from build123d import *

# Parameters (mm, degrees)
SKETCH_1_W          = 1148
SKETCH_1_H          = 195
EXTRUDE_1_DEPTH     = 15
SHELL_1_T           = -2
SKETCH_2_W          = 1148
SKETCH_2_H          = 195
SKETCH_2_W_2        = 1132
SKETCH_2_H_2        = 179
EXTRUDE_2_DEPTH     = 2
SKETCH_3_W          = 120
SKETCH_3_H          = 30
CUT_EXTRUDE_1_DEPTH = 10


with BuildPart() as part:
    # 草图1 → 凸台-拉伸1 (new body)
    with BuildSketch(Plane.XY):
        with Locations((574, 97.5)):
            Rectangle(SKETCH_1_W, SKETCH_1_H)
    extrude(amount=EXTRUDE_1_DEPTH)

    # 抽壳1
    shell_1_openings = [part.faces().sort_by_distance(p)[0] for p in [
        (574, 97.5, 15),
    ]]
    offset(amount=SHELL_1_T, openings=shell_1_openings, kind=Kind.INTERSECTION)

    # 草图2 → 凸台-拉伸2 (add)
    with BuildSketch(Plane.XY.offset(15)):
        with Locations((574, 97.5)):
            Rectangle(SKETCH_2_W, SKETCH_2_H)
        with Locations((574, 97.5)):
            Rectangle(SKETCH_2_W_2, SKETCH_2_H_2, mode=Mode.SUBTRACT)
    extrude(amount=-EXTRUDE_2_DEPTH)

    # 草图3 → 切除-拉伸1 (cut)
    with BuildSketch(Plane(origin=(0, 0, 0), x_dir=(-1, 0, 0), z_dir=(0, 0, -1))):
        with Locations((-574, 150)):
            Rectangle(SKETCH_3_W, SKETCH_3_H)
    extrude(amount=-CUT_EXTRUDE_1_DEPTH, mode=Mode.SUBTRACT)


solid = part.part
For this review, take the finished solid that the model builds, in its own axes (mm). Round coordinates to 2 decimals unless told otherwise and drop trailing zeros. Loops run counter-clockwise (first coordinate to the right, second up) from the corner with the lowest first, then second, coordinate; pieces in that order, holes last. Notation, with made-up numbers: (57, -26.5) - (69, -26.5) arc R32 ccw to (69, 12.5) - close; hole circle Ø10 at (37, 52). An arc over 180 degrees is marked (long way). Answer as CSV lines item,"result".
(1) Consider section B-B on z = 4.5. Give the boundary of the cut face in (x, y), then the cut area to 3 significant figures.
Checked values:
outline,"(0, 0) - (1148, 0) - (1148, 195) - (0, 195) - close; hole (2, 2) - (1146, 2) - (1146, 193) - (2, 193) - close"
area,"5,360 mm2"
(2) Mouldability with a two-part tool opening along X and no side actions: class faces 1 (the face through (571, 190, 13)), 2 (the face through (566, 99, 0)) as +X half, -X half, draft (parallel to the pull), parting line (faces both ways), or undercut.
Checked values:
face 1,"undercut"
face 2,"draft"
(3) Consider section C-C on y = 71. Give the boundary of the cut face in (x, z).
Checked values:
outline,"(0, 0) - (1148, 0) - (1148, 15) - (1140, 15) - (1140, 13) - (1146, 13) - (1146, 2) - (2, 2) - (2, 13) - (8, 13) - (8, 15) - (0, 15) - close"
(4) Consider section A-A on x = 586.5. Give the boundary of the cut face in (y, z).
Checked values:
outline,"(0, 0) - (135, 0) - (135, 2) - (2, 2) - (2, 13) - (8, 13) - (8, 15) - (0, 15) - close; (165, 0) - (195, 0) - (195, 15) - (187, 15) - (187, 13) - (193, 13) - (193, 2) - (165, 2) - close"
(5) Insertion check: P1, Ø2, axis at x = 913, y = 138, coming from the +Z side. The pin has a flat end and moves straight along its axis. Give the tip position at first contact, or say it passes through.
Checked values:
P1,"stops at z = 2"
(6) Consider section D-D on x = 380.5. Give the boundary of the cut face in (y, z).
Checked values:
outline,"(0, 0) - (195, 0) - (195, 15) - (187, 15) - (187, 13) - (193, 13) - (193, 2) - (2, 2) - (2, 13) - (8, 13) - (8, 15) - (0, 15) - close"
(7) Wall thickness on line 1 (Y direction, x = 941.5, z = 9); line 2 (X direction, y = 124, z = 13.75); line 3 (X direction, y = 166, z = 11.25): over which ranges is each line inside the solid? List them lowest first.
Checked values:
line 1,"y = 0 to 2, 193 to 195"
line 2,"x = 0 to 8, 1140 to 1148"
line 3,"x = 0 to 2, 1146 to 1148"
